Read the model definition and answer for the solid it produces. Units are mm, in the model's axes. A direction names the side the tool comes from. Give positions to 0.01 mm unless a question says otherwise; leave off trailing zeros. Loops run counter-clockwise (first coordinate to the right, second up) from the corner with the lowest first, then second, coordinate; pieces in that order, holes last.
(1) Determine the mould class of faces 3 (the face through (15, 0, 2)), 4 (the face through (15, 25, 2)), 5 (the face through (-5.381, 28.085, 2.535)), 6 (the face through (0, 37, 2)) for opening direction Y: pulls with the +Y half, pulls with the -Y half, needs draft (parallel to the pull), parting line crosses it, or undercut.
(2) Straight lines are drawn through the part: probe 1 along Y at (x, z) = (40, 2); probe 2 along X at (y, z) = (27, 3.7); probe 3 along X at (y, z) = (35.5, 3.1). For each, find the intervals that lie inside material, in ascending order.
(3) Find section C-C, the plane z = 1.35. Write down the section's boundary in (x, y), then the cut area to 3 significant figures.
(4) Each of these flat-tipped pins is pushed along its axis until it touches: P1, Ø3, axis at x = 38.5, y = 4, coming from the -Z side (1 decimal); P2, Ø2.5, axis at y = 38.5, z = 3.5, coming from the +X side; P3, Ø1, axis at x = 35.5, z = 0.5, coming from the -Y side. Where does it stop, or does it pass through?
(5) Find section A-A, the plane x = -10. Write down the section's boundary in (y, z).
(6) Which of the six approach directions +Z, -Z, +X, -X, +Y, -Y give full straight-line access (tool end or side, diameter ignored) to faces 1 (the face through (15, 20, 5)), 2 (the face through (3.01, 27.85, 2.46))?
(7) Find section D-D, the plane x = 14. Write down the section's boundary in (y, z), then the cut area to 3 significant figures.
(8) Find section B-B, the plane y = 17. Write down the section's boundary in (x, z).
```python
from build123d import *

# Parameters (mm, degrees)
BRACKET_PLATE_DEPTH      = 5
MOUNTING_HOLE_A_SKETCH_R = 5
MOUNTING_HOLE_A_10_DEPTH = 5
MOUNTING_HOLE_B_SKETCH_R = 5
MOUNTING_HOLE_B_10_DEPTH = 5
CORNER_FILLETS_R5_R      = 5


with BuildPart() as part:
    # Bracket Profile Sketch → Bracket Plate (new body)
    with BuildSketch(Plane.XY):
        with BuildLine():
            Line((0, 0), (30, 0))
            Line((30, 0), (50, 20))
            Line((50, 20), (50, 40))
            Line((50, 40), (30, 40))
            Line((30, 40), (30, 35))
            ThreePointArc((30, 35), (27.071067812, 27.928932188), (20, 25))
            Line((20, 25), (10, 25))
            ThreePointArc((10, 25), (2.928932188, 27.928932188), (0, 35))
            Line((0, 35), (0, 40))
            Line((0, 40), (-20, 40))
            Line((-20, 40), (-20, 20))
            Line((-20, 20), (0, 0))
        make_face()
    extrude(amount=BRACKET_PLATE_DEPTH)

    # Mounting Hole A Sketch → Mounting Hole A Ø10 (cut)
    with BuildSketch(Plane.XY.offset(5)):
        with Locations((-10, 30)):
            Circle(MOUNTING_HOLE_A_SKETCH_R)
    extrude(amount=-MOUNTING_HOLE_A_10_DEPTH, mode=Mode.SUBTRACT)

    # Mounting Hole B Sketch → Mounting Hole B Ø10 (cut)
    with BuildSketch(Plane.XY.offset(5)):
        with Locations((40, 31.609469521)):
            Circle(MOUNTING_HOLE_B_SKETCH_R)
    extrude(amount=-MOUNTING_HOLE_B_10_DEPTH, mode=Mode.SUBTRACT)

    # Corner Fillets R5
    corner_fillets_r5_edges = [part.edges().sort_by_distance(p)[0] for p in [
        (-20, 40, 2.5),
        (50, 40, 2.5),
    ]]
    fillet(corner_fillets_r5_edges, radius=CORNER_FILLETS_R5_R)


solid = part.part
```
Entries:
1. face 3: pulls with the -Y half
1. face 4: pulls with the +Y half
1. face 5: undercut
1. face 6: needs draft
2. probe 1: y = 10 to 26.61, 36.61 to 40
2. probe 2: x = -20 to -14, -6 to 4, 26 to 38.06, 41.94 to 50
2. probe 3: x = -19.97 to 0, 30 to 36.86, 43.14 to 49.97
3. outline: (-20, 20) - (0, 0) - (30, 0) - (50, 20) - (50, 35) arc R5 ccw to (45, 40) - (30, 40) - (30, 35) arc R10 cw to (20, 25) - (10, 25) arc R10 cw to (0, 35) - (0, 40) - (-15, 40) arc R5 ccw to (-20, 35) - close; hole circle Ø10 at (-10, 30); hole circle Ø10 at (40, 31.61)
3. area: 1,830 mm2
4. P1: passes through
4. P2: stops at x = 49.47
4. P3: stops at y = 5
5. outline: (10, 0) - (25, 0) - (25, 5) - (10, 5) - close; (35, 0) - (40, 0) - (40, 5) - (35, 5) - close
6. face 1: +Z, +X, -X, +Y, -Y
6. face 2: +Z, -Z, +Y
7. outline: (0, 0) - (25, 0) - (25, 5) - (0, 5) - close
7. area: 125 mm2
8. outline: (-17, 0) - (47, 0) - (47, 5) - (-17, 5) - close
